```python
from build123d import *

# Parameters (mm, degrees)
SKETCH2_R           = 7
BOSS_EXTRUDE1_DEPTH = 34
BOSS_EXTRUDE2_DEPTH = 5
SKETCH6_R           = 8
BOSS_EXTRUDE3_DEPTH = 18
SKETCH4_R           = 5
CUT_EXTRUDE1_DEPTH  = 59.460100353
CHAMFER1_SIZE       = 1
CHAMFER1_SIZE2      = 1.732050808
CHAMFER3_SIZE       = 0.5
FILLET1_R           = 0.5


with BuildPart() as part:
    # Sketch2 → Boss-Extrude1 (new body)
    with BuildSketch(Plane(origin=(0, 0, 0), x_dir=(1, 0, 0), z_dir=(0, 1, 0))):
        with Locations(Location((0, 0, 0), (0, 0, 270))):
            Circle(SKETCH2_R)
    extrude(amount=BOSS_EXTRUDE1_DEPTH)

    # Sketch3 → Cut-Revolve1 (revolve, cut)
    with BuildSketch(Plane.XY, mode=Mode.PRIVATE) as cut_revolve1_sk:
        Polygon((6.5, 34), (7, 32), (6.5, 32), (6.5, 29.5), (7, 27.5), (6.5, 27.5), (6.5, 25), (7, 23), (6.5, 23), (6.5, 20.5), (7, 18.5), (7, 34), align=None)
    revolve(cut_revolve1_sk.sketch.rotate(Axis((0, 0, 0), (0, 1, 0)), 90), axis=Axis((0, 0, 0), (0, 1, 0)), mode=Mode.SUBTRACT)

    # Sketch5 → Boss-Extrude2 (add)
    with BuildSketch(Plane.XZ):
        Polygon((8.5, -4.907477288), (8.5, 4.907477288), (0, 9.814954576), (-8.5, 4.907477288), (-8.5, -4.907477288), (0, -9.814954576), align=None)
    extrude(amount=BOSS_EXTRUDE2_DEPTH)

    # Sketch6 → Boss-Extrude3 (add)
    with BuildSketch(Plane.XZ.offset(5)):
        with Locations(Location((0, 0, 0), (0, 0, 270))):
            Circle(SKETCH6_R)
    extrude(amount=BOSS_EXTRUDE3_DEPTH)

    # Sketch4 → Cut-Extrude1 (cut, through all)
    with BuildSketch(Plane(origin=(0, 34, 0), x_dir=(1, 0, 0), z_dir=(0, 1, 0))):
        with Locations(Location((0, 0, 0), (0, 0, 270))):
            Circle(SKETCH4_R)
    extrude(amount=-CUT_EXTRUDE1_DEPTH, mode=Mode.SUBTRACT)

    # Chamfer1
    chamfer1_edges = [part.edges().sort_by_distance(p)[0] for p in [
        (4.25, 0, -7.361215932),
        (8.5, 0, 0),
        (4.25, 0, 7.361215932),
        (-4.25, 0, 7.361215932),
        (-8.5, 0, 0),
        (-4.25, 0, -7.361215932),
    ]]
    chamfer1_side = [part.faces().sort_by_distance(p)[0] for p in [
        (8.240320711, 0, 0),
    ]]
    chamfer(chamfer1_edges, length=CHAMFER1_SIZE, length2=CHAMFER1_SIZE2, reference=chamfer1_side[0])

    # Chamfer3
    chamfer3_edges = [part.edges().sort_by_distance(p)[0] for p in [
        (0, -23, 8),
    ]]
    chamfer(chamfer3_edges, length=CHAMFER3_SIZE)

    # Fillet1
    fillet1_edges = [part.edges().sort_by_distance(p)[0] for p in [
        (0, 34, 6.5),
    ]]
    fillet(fillet1_edges, radius=FILLET1_R)


solid = part.part
```
Source: CAD feature listing. Evaluate the final solid. Frame: model axes, mm. A direction names the side the tool comes from. Round coordinates to 2 decimals unless told otherwise and drop trailing zeros. Loops run counter-clockwise (first coordinate to the right, second up) from the corner with the lowest first, then second, coordinate; pieces in that order, holes last. Notation, with made-up numbers: M 67,-33 L 77,-33 A21 ccw 77,-11 Z; hole C 60,50.25 d3. An arc over 180 degrees is marked long. Use a Markdown table: item, result. Add a question column.
1. Mould query, pull axis Y, two halves, no side actions, for faces 1 (the flat face through (-8.5, -3, 0)), 2 (the flat face through (-3.94, -0.88, 6.97)), 3 (the cylindrical face through (3.955, 30.732, 5.158)). Classes: pulls with the +Y half, pulls with the -Y half, needs draft (parallel to the pull), parting line crosses it, or undercut.
2. Reachability of faces 4 (the flat face through (4.191, -3.343, -7.396)), 5 (the cylindrical face through (-7.81, -13.63, 1.73)), 6 (the cylindrical face through (3.955, 21.732, 5.158)) from +Z, -Z, +X, -X, +Y, -Y: full face, straight path, thin tool, end or side. Return the list, or none.
3. Contact query for flat-ended pins moving along their axis: P1, Ø4, axis at y = 13, z = -3, coming from the +X side; P2, Ø5, axis at x = -0.5, y = 10.5, coming from the -Z side; P3, Ø1.5, axis at x = 4, y = -16.5, coming from the -Z side. Output: stop coordinate, or through.
4. Section query A-A on y = 22. Return the cut outline in (x, z), then the cut area to 3 significant figures.
5. Line query: line 1 (X direction, y = 11, z = 0); line 2 (X direction, y = -3.5, z = 0); line 3 (Z direction, x = -1.5, y = 27). Output: solid intervals per line, ascending.
Reported:
| question | item | result |
|---|---|---|
| 1 | face 1 | needs draft |
| 1 | face 2 | pulls with the +Y half |
| 1 | face 3 | undercut |
| 2 | face 4 | -Z, +X, +Y, -Y |
| 2 | face 5 | -Y |
| 2 | face 6 | none |
| 3 | P1 | stops at x = 6.93 |
| 3 | P2 | stops at z = -7 |
| 3 | P3 | stops at z = -7.31 |
| 4 | outline | C 0,0 d13; hole C 0,0 d10 |
| 4 | area | 54.2 mm² |
| 5 | line 1 | x = -7 to -5, 5 to 7 |
| 5 | line 2 | x = -8.5 to -5, 5 to 8.5 |
| 5 | line 3 | z = -6.32 to -4.77, 4.77 to 6.32 |
